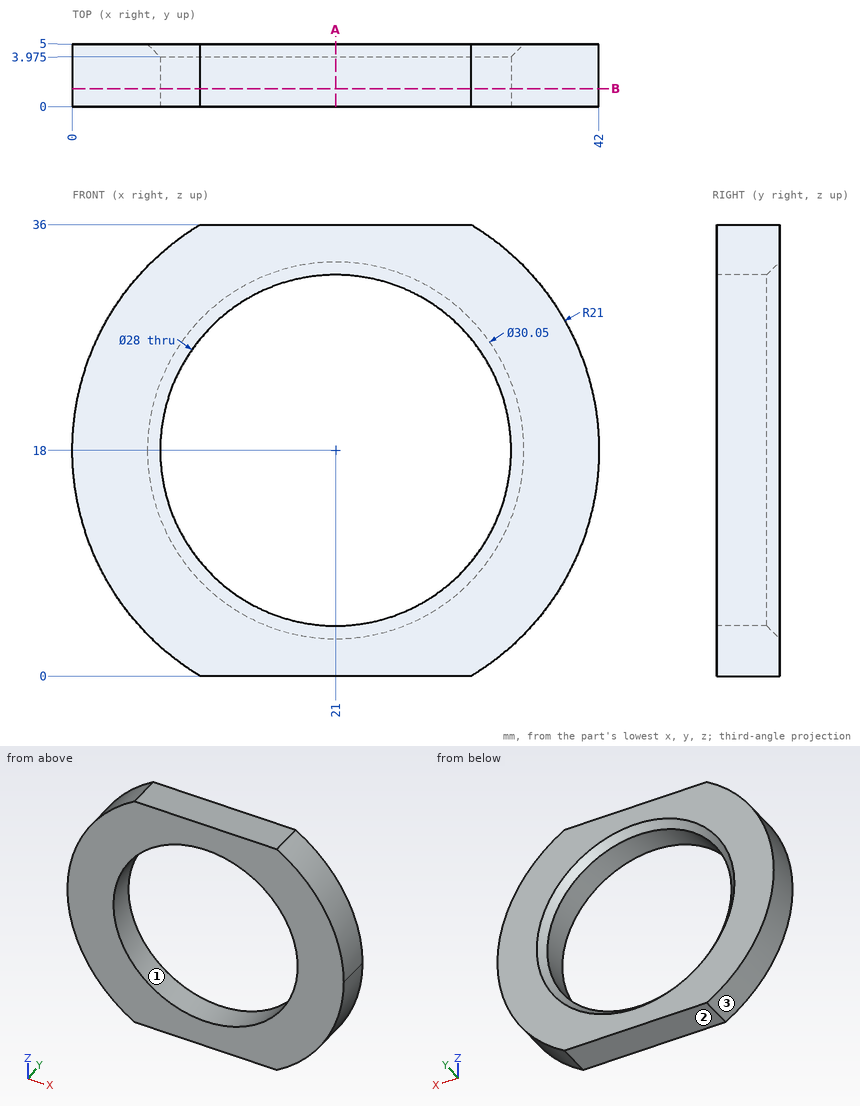
Check sheet for the drawn part. Datum: minimum x, y, z corner. Units: mm. Give positions to 0.01 mm unless a question says otherwise; leave off trailing zeros. Order: outer loops, then holes, each group sorted by start corner. A loop starts at its lowest first (then second) coordinate and runs counter-clockwise, first axis right, second up. Notation, with made-up numbers: (47, 13) - (90, 13) arc R19 cw to (90, 47) - close; hole circle Ø6 at (78.25, 52.25). An arc over 180 degrees is marked (long way). Write item = value, one per line. Start each with the question number.
1) Section check B-B (y = 1.45). Enter the section's corners in (x, z), then the cut area to 3 significant figures.
2) Scan lines: L1, parallel to Z at x = 21, y = 0.9; L2, parallel to X at y = 2.15, z = 25.5; L3, parallel to X at y = 3.15, z = 12. Record each from-to range of solid material in increasing order.
3) Gauge pin test, flat ends, axial feed: pin 1 Ø3 at (x, z) = (23, 7.5) entering from +Y; pin 2 Ø2 at (x, y) = (37, 2) entering from -Z; pin 3 Ø1.5 at (y, z) = (1.5, 6.5) entering from -X. Record the tip position at first contact, or that the pin passes through.
4) Section check A-A (x = 21). Enter the section's corners in (y, z) (3 decimals), then the cut area to 3 significant figures.
5) Draft check along Z on the marked faces 1, 2 and 3. Enter one of: released by +Z, released by -Z, zero draft, split by the parting line, or undercut.
Geometry check:
q1.outline = (10.18, 0) - (31.82, 0) arc R21 ccw to (31.82, 36) - (10.18, 36) arc R21 ccw to start; hole circle Ø28 at (21, 18)
q1.area = 682 mm2
q2.L1 = 0 to 4, 32 to 36
q2.L2 = 1.38 to 9.18, 32.82 to 40.62
q2.L3 = 0.88 to 8.35, 33.65 to 41.12
q3.pin_1 = through
q3.pin_2 = 3.3
q3.pin_3 = 2.96
q4.outline = (0, 0) - (5, 0) - (5, 2.975) - (3.975, 4) - (0, 4) - close; (0, 32) - (3.975, 32) - (5, 33.025) - (5, 36) - (0, 36) - close
q4.area = 38.9 mm2
q5.face_1 = undercut
q5.face_2 = released by -Z
q5.face_3 = split by the parting line
